CAD build for the part. Positions are in the model's coordinates, mm. Give positions to 0.01 mm unless a question says otherwise; leave off trailing zeros. Order: outer loops, then holes, each group sorted by start corner. A loop starts at its lowest first (then second) coordinate and runs counter-clockwise, first axis right, second up. Notation, with made-up numbers: (-32.75, 13) -> (0.25, 13) arc R23 cw to (0.25, 29) -> close; hole circle Ø10 at (45, 75). An arc over 180 degrees is marked (long way). Use one line per item in the form item = value. Start each with the question number.
1) Mould opens along Y. For faces 1 (the face through (59, -3, 2)), 2 (the face through (158.6, 12.9, 1)), 3 (the face through (-47.957, -2.038, 0.986)) say: pulls with the +Y half, pulls with the -Y half, needs draft (parallel to the pull), parting line crosses it, or undercut.
2) Cut at C-C, the plane z = 1.6. Give the cut face in (x, y).
3) Probe line 1 (Y direction, x = 58.79, z = 0.9); line 2 (Y direction, x = 117.58, z = 0.85); line 3 (X direction, y = 26, z = 1.8). List the from-to ranges inside material, lowest first.
4) Cut at B-B, the plane y = 0. Give the cut face in (x, z).
5) Drop flat-ended pins along their axis: P1, Ø1, axis at y = 29, z = 1.5, coming from the -X side; P2, Ø0.6, axis at x = 60.5, z = 1.5, coming from the -Y side; P3, Ø4.5, axis at x = 58.79, y = 0, coming from the +Z side; P4, Ø1, axis at y = 2.5, z = 1, coming from the +X side. Give the stop position or say it passes through.
6) Cut at A-A, the plane x = 117.58. Give the cut face in (y, z), and give its area (3 significant figures).
7) Cut at D-D, the plane x = 58.79. Give the cut face in (y, z).
from build123d import *

# Parameters (mm, degrees)
SKETCH1_R           = 43
SKETCH1_R_2         = 2.5
BOSS_EXTRUDE1_DEPTH = 2


with BuildPart() as part:
    # Sketch1 → Boss-Extrude1 (new body)
    with BuildSketch(Plane.XY):
        with BuildLine():
            Line((47.617811618, 6.045164742), (69.962188382, 6.045164742))
            ThreePointArc((69.962188382, 6.045164742), (165.579998377, -0.012483332), (69.959050499, -6.020396052))
            Line((69.959050499, -6.020396052), (47.620949501, -6.020396052))
            ThreePointArc((47.620949501, -6.020396052), (-47.999998377, -0.012483332), (47.617811618, 6.045164742))
        make_face()
        Circle(SKETCH1_R, mode=Mode.SUBTRACT)
        with Locations((117.58, 0)):
            Circle(SKETCH1_R, mode=Mode.SUBTRACT)
        with Locations((58.79, 0)):
            Circle(SKETCH1_R_2, mode=Mode.SUBTRACT)
    extrude(amount=BOSS_EXTRUDE1_DEPTH)


solid = part.part
Result:
q1.face_1 = needs draft
q1.face_2 = undercut
q1.face_3 = parting line crosses it
q2.outline = (47.62, -6.02) -> (69.96, -6.02) arc R48 ccw (long way) to (69.96, 6.05) -> (47.62, 6.05) arc R48 ccw (long way) to start; hole circle Ø86 at (0, 0); hole circle Ø5 at (58.79, 0); hole circle Ø86 at (117.58, 0)
q3.line_1 = -6.02 to -2.5, 2.5 to 6.05
q3.line_2 = -48 to -43, 43 to 48
q3.line_3 = -40.35 to -34.25, 34.25 to 40.35, 77.23 to 83.33, 151.83 to 157.93
q4.outline = (-48, 0) -> (-43, 0) -> (-43, 2) -> (-48, 2) -> close; (43, 0) -> (56.29, 0) -> (56.29, 2) -> (43, 2) -> close; (61.29, 0) -> (74.58, 0) -> (74.58, 2) -> (61.29, 2) -> close; (160.58, 0) -> (165.58, 0) -> (165.58, 2) -> (160.58, 2) -> close
q5.P1 = -38.62
q5.P2 = -6.02
q5.P3 = through
q5.P4 = 165.54
q6.outline = (-48, 0) -> (-43, 0) -> (-43, 2) -> (-48, 2) -> close; (43, 0) -> (48, 0) -> (48, 2) -> (43, 2) -> close
q6.area = 20.0 mm²
q7.outline = (-6.02, 0) -> (-2.5, 0) -> (-2.5, 2) -> (-6.02, 2) -> close; (2.5, 0) -> (6.05, 0) -> (6.05, 2) -> (2.5, 2) -> close
